Could you check a few things on this model? Use its own coordinates, in mm. A direction names the side the tool comes from. Give positions to 0.01 mm unless a question says otherwise; leave off trailing zeros. Order: outer loops, then holes, each group sorted by start corner. A loop starts at its lowest first (then second) coordinate and runs counter-clockwise, first axis right, second up. Notation, with made-up numbers: (11, 82) -> (31, 82) arc R21 ccw to (31, 118) -> close; hole circle Ø1 at (86.25, 10). An arc over 180 degrees is marked (long way). Write each question's results on one line, items separated by ' | '.
```python
from build123d import *

# Parameters (mm, degrees)
MEMBER_1_DEPTH      = 76
SKETCH_4_R          = 23
CUT_EXTRUDE_1_DEPTH = 171.223382648
SKETCH_6_R          = 4.5
CUT_EXTRUDE_2_DEPTH = 171.223382648
HOLE_WIZARD_M6_1_D  = 5


with BuildPart() as part:
    # Sketch11 → Member 1 (new body)
    with BuildSketch(Plane(origin=(0, 0, 0), x_dir=(0, 0, -1), z_dir=(1, 0, 0))):
        with BuildLine():
            Line((60, 140), (0, 140))
            Line((0, 140), (0, 0))
            Line((0, 0), (60, 0))
            Line((60, 0), (60, 1.539529212))
            ThreePointArc((60, 1.539529212), (58.844151715, 4.550616941), (55.970378085, 6.014877742))
            Line((55.970378085, 6.014877742), (15.163772294, 10.303824837))
            ThreePointArc((15.163772294, 10.303824837), (10.054841396, 12.906955149), (8, 18.26))
            Line((8, 18.26), (8, 121.74))
            ThreePointArc((8, 121.74), (10.054841396, 127.093044851), (15.163772294, 129.696175163))
            Line((15.163772294, 129.696175163), (55.970378085, 133.985122258))
            ThreePointArc((55.970378085, 133.985122258), (58.844151715, 135.449383059), (60, 138.460470788))
            Line((60, 138.460470788), (60, 140))
        make_face()
    extrude(amount=MEMBER_1_DEPTH)

    # 草图4 → 切除-拉伸1 (cut, through all)
    with BuildSketch(Plane.XY):
        with Locations((38, 70)):
            Circle(SKETCH_4_R)
    extrude(amount=-CUT_EXTRUDE_1_DEPTH, mode=Mode.SUBTRACT)

    # 草图6 → 切除-拉伸2 (cut, through all)
    with BuildSketch(Plane.XY):
        with Locations((66.25, 41.75)):
            Circle(SKETCH_6_R)
        with Locations((9.75, 41.75)):
            Circle(SKETCH_6_R)
        with Locations((66.25, 98.25)):
            Circle(SKETCH_6_R)
        with Locations((9.75, 98.25)):
            Circle(SKETCH_6_R)
    extrude(amount=-CUT_EXTRUDE_2_DEPTH, mode=Mode.SUBTRACT)

    # M6 螺纹孔1 (through all)
    with Locations(Plane(origin=(0, 0, 0), x_dir=(-1, 0, 0), z_dir=(0, -1, 0))):
        with Locations((-65.5, 15), (-65.5, 45), (-10.5, 15), (-10.5, 45)):
            Hole(HOLE_WIZARD_M6_1_D / 2)


solid = part.part
```
Q1. I need wall thicknesses on line 1 along X through (y, z) = (137, -45); line 2 along Y through (x, z) = (9.75, -2.5); line 3 along Z through (x, y) = (10.5, 137.5). Which ranges of each line are inside material? Lowest first, please.
Here are the results:
line 1: x = 0 to 8, 13 to 63, 68 to 76 | line 2: y = 0 to 37.25, 46.25 to 93.75, 102.75 to 140 | line 3: z = -59.9 to -47.5, -42.5 to -17.5, -12.5 to 0
Q2. Suppose I cut it at C-C on z = -45. Please give me the cut outline in (x, y).
Here are the results:
outline: (0, 0) -> (8, 0) -> (8, 7.17) -> (0, 7.17) -> close; (0, 132.83) -> (8, 132.83) -> (8, 140) -> (0, 140) -> close; (13, 0) -> (63, 0) -> (63, 7.17) -> (13, 7.17) -> close; (13, 132.83) -> (63, 132.83) -> (63, 140) -> (13, 140) -> close; (68, 0) -> (76, 0) -> (76, 7.17) -> (68, 7.17) -> close; (68, 132.83) -> (76, 132.83) -> (76, 140) -> (68, 140) -> close
Q3. Suppose I cut it at A-A on y = 70. Please give me the cut outline in (x, z), and give its area (3 significant figures).
Here are the results:
outline: (0, -8) -> (15, -8) -> (15, 0) -> (0, 0) -> close; (61, -8) -> (76, -8) -> (76, 0) -> (61, 0) -> close | area: 240 mm²
Q4. Suppose I cut it at B-B on x = 38. Please give me the cut outline in (y, z).
Here are the results:
outline: (0, -60) -> (1.54, -60) arc R4.5 ccw to (6.01, -55.97) -> (10.3, -15.16) arc R8 cw to (18.26, -8) -> (47, -8) -> (47, 0) -> (0, 0) -> close; (93, -8) -> (121.74, -8) arc R8 cw to (129.7, -15.16) -> (133.99, -55.97) arc R4.5 ccw to (138.46, -60) -> (140, -60) -> (140, 0) -> (93, 0) -> close
Q5. Thinking about a two-plate mould opening in X: for faces 1 (the flat face through (37.47, 8.13, -35.85)), 2 (the flat face through (0, 65.1, -7.6)), 3 (the cylindrical face through (68.669, 102.044, -3.944)), which applies, +X half, -X half, draft (parallel to the pull), parting line (faces both ways), or undercut?
Here are the results:
face 1: draft | face 2: -X half | face 3: undercut
Q6. Suppose I cut it at D-D on y = 100.5. Please give me the cut outline in (x, z).
Here are the results:
outline: (0, -8) -> (5.85, -8) -> (5.85, 0) -> (0, 0) -> close; (13.65, -8) -> (62.35, -8) -> (62.35, 0) -> (13.65, 0) -> close; (70.15, -8) -> (76, -8) -> (76, 0) -> (70.15, 0) -> close
Q7. I'm going to push a flat-ended pin straight in: pin 1 Ø12 at (x, y) = (58.5, 76.5) entering from -Z. Where does the tip first touch, or does it pass through?
Here are the results:
pin 1: stops at z = -8
Q8. For faces 4 (the cylindrical face through (37.468, 12.846, -10.11)), 5 (the flat face through (76, 65.1, -7.6)), which set-ups out of +Z, -Z, +X, -X, +Y, -Y let a thin tool reach every point of the face, with its end or its side?
Here are the results:
face 4: -Z, +X, -X | face 5: +Z, -Z, +X, +Y, -Y
